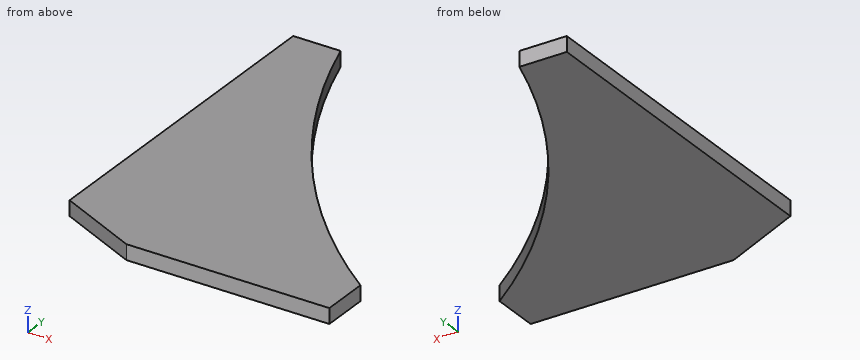
```python
from build123d import *

# Parameters (mm, degrees)
BOSS_EXTRUDE1_DEPTH = 4
CHAMFER1_SIZE       = 20
CHAMFER1_SIZE2      = 43
CUT_EXTRUDE1_DEPTH  = 10


with BuildPart() as part:
    # Sketch1 → Boss-Extrude1 (new, symmetric)
    with BuildSketch(Plane.XY):
        Polygon((0, 0), (150, 0), (150, 25), (25, 200), (0, 200), align=None)
    extrude(amount=BOSS_EXTRUDE1_DEPTH, both=True)

    # Chamfer1
    chamfer1_edges = [part.edges().sort_by_distance(p)[0] for p in [
        (0, 0, 0),
    ]]
    chamfer1_side = [part.faces().sort_by_distance(p)[0] for p in [
        (0, 100, 0),
    ]]
    chamfer(chamfer1_edges, length=CHAMFER1_SIZE, length2=CHAMFER1_SIZE2, reference=chamfer1_side[0])

    # Sketch2 → Cut-Extrude1 (cut)
    with BuildSketch(Plane.XY.offset(4)):
        with BuildLine():
            ThreePointArc((25, 200), (73.72578288, 102.661273486), (150, 25))
            Line((150, 25), (25, 200))
        make_face()
    extrude(amount=-CUT_EXTRUDE1_DEPTH, mode=Mode.SUBTRACT)


solid = part.part
```
Geometry: final body of the model. Coordinates: model frame, mm. Give positions to 0.01 mm unless a question says otherwise; leave off trailing zeros. Loops run counter-clockwise (first coordinate to the right, second up) from the corner with the lowest first, then second, coordinate; pieces in that order, holes last. Notation, with made-up numbers: (52, 67) -> (82, 67) arc R20 cw to (82, 106) -> close; hole circle Ø3 at (-23, 17.5). An arc over 180 degrees is marked (long way). Return JSON: item names as keys, results as strings.
Item 1: Section A-A, the plane z = -1.5. Output: boundary loops of the cut face in (x, y).
Filled in:
{"outline": "(0, 20) -> (43, 0) -> (150, 0) -> (150, 25) arc R350 cw to (25, 200) -> (0, 200) -> close"}
Item 2: Section C-C, the plane x = 103. Output: boundary loops of the cut face in (y, z).
Filled in:
{"outline": "(0, -4) -> (66.92, -4) -> (66.92, 4) -> (0, 4) -> close"}
Item 3: Section B-B, the plane y = 137. Output: boundary loops of the cut face in (x, z).
Filled in:
{"outline": "(0, -4) -> (52.09, -4) -> (52.09, 4) -> (0, 4) -> close"}
Item 4: Pin query (flat end, axial travel): P1, Ø3, axis at x = 39, z = 2.5, coming from the +Y side; P2, Ø2, axis at x = 61.5, z = -1, coming from the +Y side; P3, Ø1, axis at y = 26.5, z = -1.5, coming from the +X side. Return the tip coordinate at first contact, or that it passes through.
Filled in:
{"P1": "y = 166.67", "P2": "y = 122.58", "P3": "x = 148.66"}
Item 5: Line query: line 1 (X direction, y = 88, z = 3.5); line 2 (Y direction, x = 134, z = 0.5); line 3 (X direction, y = 103.5, z = 0.5). Output: solid intervals per line, ascending.
Filled in:
{"line 1": "0 to 84.79", "line 2": "0 to 37.61", "line 3": "0 to 73.13"}
